The figure shows three views and two pictorial views of one solid part (mm, origin at its lowest corner). Answer the questions. A direction names the side the tool comes from. Give positions to 0.01 mm unless a question says otherwise; leave off trailing zeros. Order: outer loops, then holes, each group sorted by start corner. A loop starts at its lowest first (then second) coordinate and runs counter-clockwise, first axis right, second up. Notation, with made-up numbers: (89.25, 31) - (146.25, 31) arc R10 cw to (146.25, 38) - close; hole circle Ø1 at (69.25, 16.5). An arc over 180 degrees is marked (long way). Use a Markdown table: item, result. Add a question column.
1. A cutting plane is placed at A-A on x = 7.5. Determine the outline of the cut face in (y, z) (1 decimal), and give its area (3 significant figures).
2. A cutting plane is placed at B-B on y = 7. Determine the outline of the cut face in (x, z).
3. Flat-ended cylindrical pins translate along their axes: P1, Ø5, axis at y = 5, z = 7, coming from the +X side; P2, Ø1.5, axis at y = 1.5, z = 6, coming from the -X side; P3, Ø1, axis at y = 10.5, z = 21.5, coming from the +X side; P4, Ø4, axis at y = 10, z = 9, coming from the -X side. Find the tip coordinate at first contact, or state that the pin passes through.
4. Which of the six approach directions +Z, -Z, +X, -X, +Y, -Y give full straight-line access (tool end or side, diameter ignored) to the marked faces 1 and 2?
5. A cutting plane is placed at D-D on z = 19.25. Determine the outline of the cut face in (x, y) (1 decimal).
6. Consider L1, parallel to Z at x = 5.5, y = 2.75; L2, parallel to X at y = 6.5, z = 14.75; L3, parallel to X at y = 8, z = 16.25 (1 decimal). Determine where each line is inside the solid, lowest interval first.
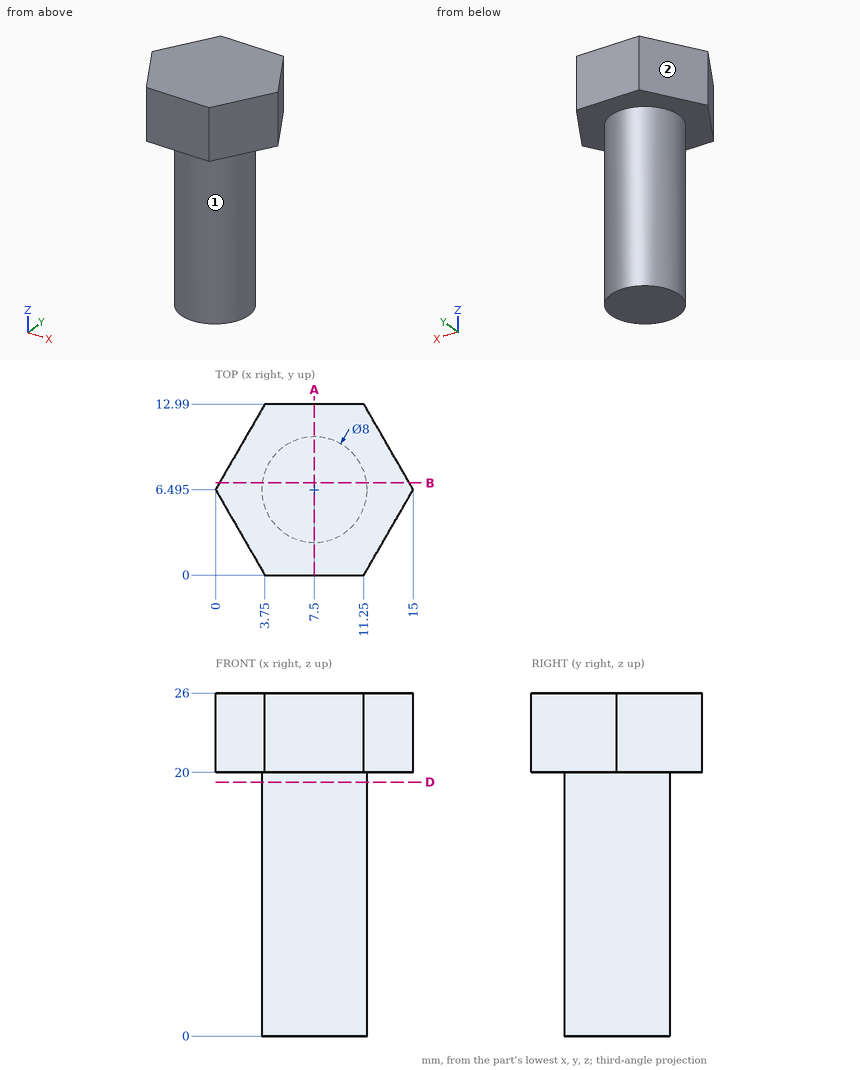
Output values:
| question | item | result |
|---|---|---|
| 1 | outline | (0, 20) - (2.5, 20) - (2.5, 0) - (10.5, 0) - (10.5, 20) - (13, 20) - (13, 26) - (0, 26) - close |
| 1 | area | 238 mm² |
| 2 | outline | (0.29, 20) - (3.53, 20) - (3.53, 0) - (11.47, 0) - (11.47, 20) - (14.71, 20) - (14.71, 26) - (0.29, 26) - close |
| 3 | P1 | x = 11.5 |
| 3 | P2 | through |
| 3 | P3 | x = 12.98 |
| 3 | P4 | x = 3.79 |
| 4 | face 1 | -Z |
| 4 | face 2 | +Z, -Z, -X, +Y |
| 5 | outline | circle Ø8 at (7.5, 6.5) |
| 6 | L1 | 20 to 26 |
| 6 | L2 | 3.5 to 11.5 |
| 6 | L3 | 3.8 to 11.2 |
